Drawing for the job (mm, zero at the part's lowest x, y, z). A direction names the side the tool comes from. Round coordinates to 2 decimals unless told otherwise and drop trailing zeros. Loops run counter-clockwise (first coordinate to the right, second up) from the corner with the lowest first, then second, coordinate; pieces in that order, holes last. Notation, with made-up numbers: (26.5, -21.75) - (67.5, -21.75) arc R20 cw to (67.5, -5.75) - close; hole circle Ø6 at (-3, -14). An arc over 180 degrees is marked (long way). Put each result on its own line as item: value.
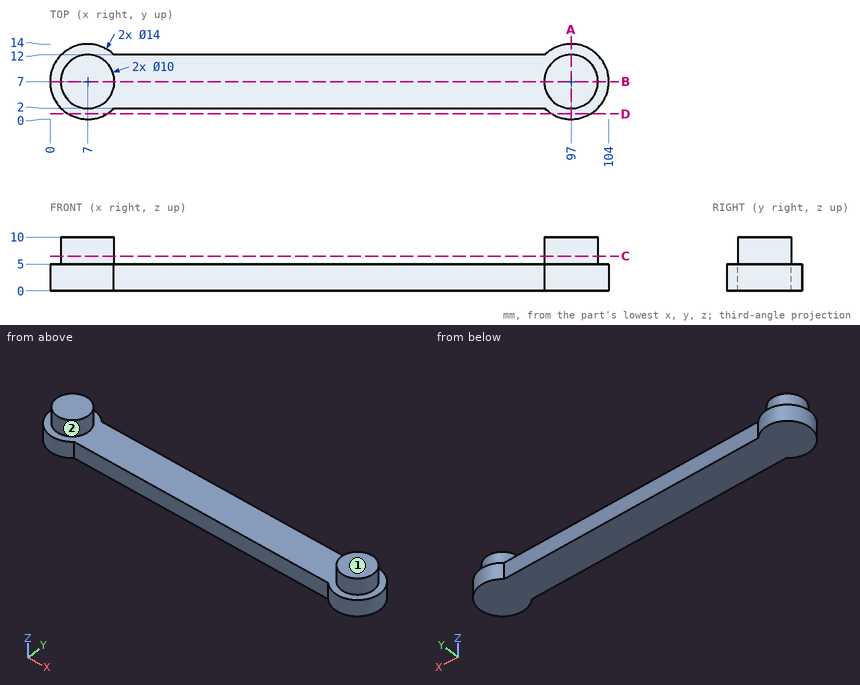
1. Band-saw the part on B-B (y = 7). List the corners of the cut face in (x, z), plus the area to 3 significant figures.
A:
outline: (0, 0) - (104, 0) - (104, 5) - (102, 5) - (102, 10) - (92, 10) - (92, 5) - (12, 5) - (12, 10) - (2, 10) - (2, 5) - (0, 5) - close
area: 620 mm²
2. Pin check, flat tips, straight feed: P1, Ø1, axis at x = 40.5, y = 9, coming from the +Z side; P2, Ø4, axis at y = 10.5, z = 5, coming from the +X side; P3, Ø1.5, axis at y = 8, z = 4, coming from the +X side. Stop position of each tip, or through.
A:
P1: stops at z = 5
P2: stops at x = 103.84
P3: stops at x = 104
3. Probe line 1 along Y through (x, z) = (28, 2.75); line 2 along Z through (x, y) = (46, 9.25); line 3 along X through (y, z) = (6.75, 6.75). List the from-to ranges inside material, lowest first. Write a range as [from, to].
A:
line 1: y = [2, 12]
line 2: z = [0, 5]
line 3: x = [2.01, 11.99], [92.01, 101.99]
4. Band-saw the part on C-C (z = 6.5). List the corners of the cut face in (x, y), plus the area to 3 significant figures.
A:
outline: circle Ø10 at (7, 7); circle Ø10 at (97, 7)
area: 157 mm²
5. Tool access for the marked faces 1 and 2: list every direction of +Z, -Z, +X, -X, +Y, -Y with a clear straight run to the whole face (end or side of a thin tool).
A:
face 1: +Z, +X, -X, +Y, -Y
face 2: +Z
6. Band-saw the part on D-D (y = 1). List the corners of the cut face in (x, z).
A:
outline: (3.39, 0) - (10.61, 0) - (10.61, 5) - (3.39, 5) - close; (93.39, 0) - (100.61, 0) - (100.61, 5) - (93.39, 5) - close
7. Band-saw the part on A-A (x = 97). List the corners of the cut face in (y, z).
A:
outline: (0, 0) - (14, 0) - (14, 5) - (12, 5) - (12, 10) - (2, 10) - (2, 5) - (0, 5) - close
